For this review, use the dimensioned drawing (mm, ordinates from the lowest corner) and the shaded views. A direction names the side the tool comes from. Coordinates: 2 decimals unless noted, no trailing zeros. Loops run counter-clockwise (first coordinate to the right, second up) from the corner with the lowest first, then second, coordinate; pieces in that order, holes last. Notation, with made-up numbers: M 20.5,-29 L 75.5,-29 A8 ccw 75.5,-17 Z; hole C 10.25,88.25 d7. An arc over 180 degrees is marked long. One line per item, written item: value.
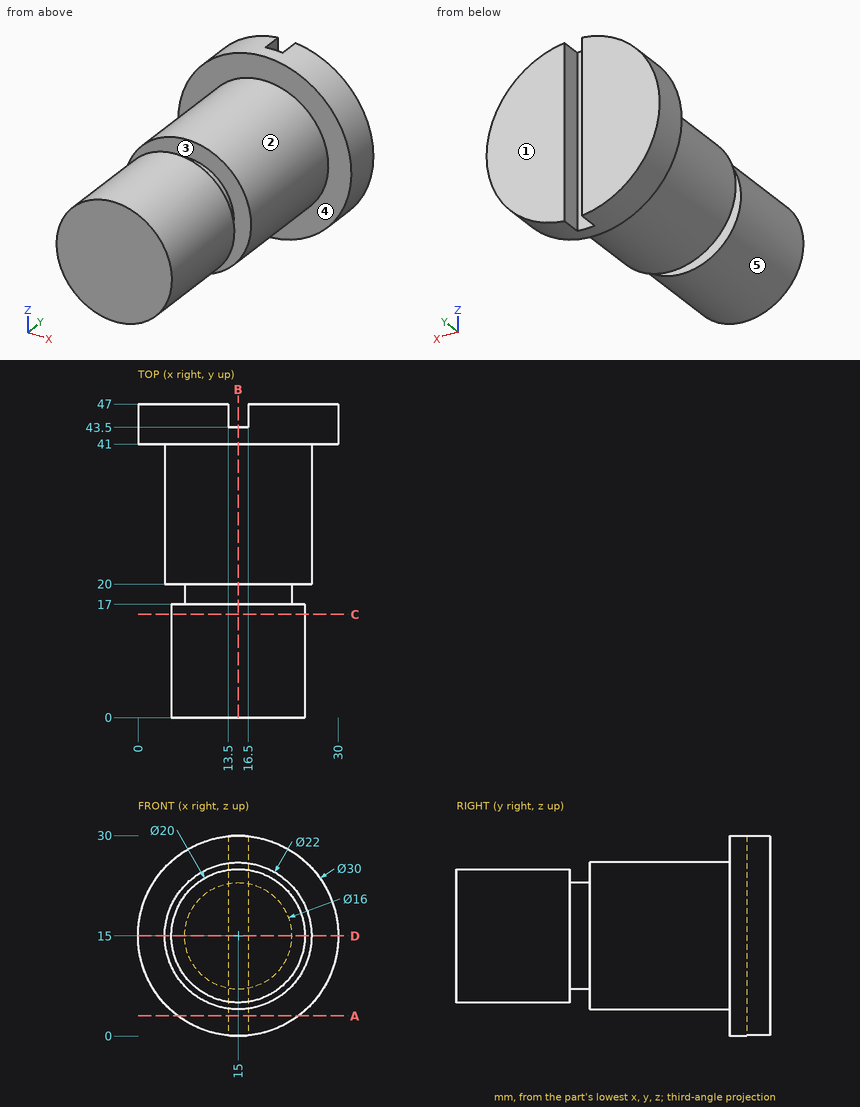
(1) We need section B-B on x = 15. State the section outline as (y, z) points.
Reply:
outline: M 0,5 L 17,5 L 17,7 L 20,7 L 20,4 L 41,4 L 41,0 L 43.5,0 L 43.5,30 L 41,30 L 41,26 L 20,26 L 20,23 L 17,23 L 17,25 L 0,25 Z
(2) To check wall thickness, follow line 1 along Y through (x, z) = (8, 8.75); line 2 along Y through (x, z) = (20, 3.75); line 3 along Y through (x, z) = (23.75, 8.75). State the ranges of each line that lie inside material, in increasing order. Write a range as [from, to].
Reply:
line 1: y = [0, 17], [20, 47]
line 2: y = [41, 47]
line 3: y = [20, 47]
(3) We need section C-C on y = 15.5. State the section outline as (x, z) points, then the cut area to 3 significant figures.
Reply:
outline: C 15,15 d20
area: 314 mm2
(4) Mouldability with a two-part tool opening along Y and no side actions: class the marked faces 3, 4 and 5 as released by +Y, released by -Y, zero draft, split by the parting line, or undercut.
Reply:
face 3: undercut
face 4: released by -Y
face 5: zero draft
(5) Tool access review of the marked faces 1 and 2: name each direction out of +Z, -Z, +X, -X, +Y, -Y from which nothing blocks a thin tool from reaching the whole face with its end or side.
Reply:
face 1: +Z, -Z, +X, -X, +Y
face 2: -Y
(6) We need section D-D on z = 15. State the section outline as (x, y) points.
Reply:
outline: M 0,41 L 4,41 L 4,20 L 7,20 L 7,17 L 5,17 L 5,0 L 25,0 L 25,17 L 23,17 L 23,20 L 26,20 L 26,41 L 30,41 L 30,47 L 16.5,47 L 16.5,43.5 L 13.5,43.5 L 13.5,47 L 0,47 Z
(7) We need section A-A on z = 3. State the section outline as (x, y) points, then the cut area to 3 significant figures.
Reply:
outline: M 6,41 L 24,41 L 24,47 L 16.5,47 L 16.5,43.5 L 13.5,43.5 L 13.5,47 L 6,47 Z
area: 97.5 mm2
(8) Insertion check: pin 1 (3 mm diameter, centred on y = 8, z = 14, fed in from -X); pin 2 (2 mm diameter, centred on x = 19, z = 27, fed in from -Y); pin 3 (1 mm diameter, centred on x = 21, y = 37, fed in from -Z). Each pin has a flat end and moves straight along its axis. Give the tip position at first contact, or say it passes through.
Reply:
pin 1: stops at x = 5
pin 2: stops at y = 41
pin 3: stops at z = 5.47
